```python
from build123d import *

# Parameters (mm, degrees)
BOSS_EXTRUDE1_DEPTH      = 10
BOSS_EXTRUDE2_DEPTH      = 10
BOSS_EXTRUDE2_DEPTH_BACK = 26
SKETCH2_R                = 5.820264096
CUT_EXTRUDE1_DEPTH       = 629.17046577
CUT_EXTRUDE1_DEPTH_BACK  = 629.17046577
SKETCH3_R                = 7.5


with BuildPart() as part:
    # Sketch1 → Boss-Extrude1 (new body)
    with BuildSketch(Plane.XY):
        with BuildLine():
            Line((-267.317020812, 384.57192575), (-267.301609192, 354.315771574))
            ThreePointArc((-267.301609192, 354.315771574), (-464.45214838, 194.902560898), (-291.585214163, 9.435771703))
            Line((-291.585214163, 9.435771703), (-291.585214163, -20.564228297))
            ThreePointArc((-291.585214163, -20.564228297), (-494.516390011, 194.886544), (-267.317020812, 384.57192575))
        make_face()
    extrude(amount=-BOSS_EXTRUDE1_DEPTH)

    # Sketch2 → Boss-Extrude2 (add, two sides: drawn at the far end of the back side and taken through both)
    with BuildSketch(Plane.XY.offset(-BOSS_EXTRUDE2_DEPTH_BACK)):
        with Locations((-307.201523558, -4.519874966)):
            Circle(SKETCH2_R)
    extrude(amount=BOSS_EXTRUDE2_DEPTH + BOSS_EXTRUDE2_DEPTH_BACK)

    # Sketch3 → Cut-Extrude1 (cut, two sides: drawn at the far end of the back side and taken through both)
    with BuildSketch(Plane.XY.offset(-CUT_EXTRUDE1_DEPTH_BACK)):
        with Locations(Location((-421.223956701, 321.632808197, 0), (0, 0, 180))):
            Circle(SKETCH3_R)
        with Locations(Location((-353.128945359, 362.487113382, 0), (0, 0, 180))):
            Circle(SKETCH3_R)
        with BuildLine():
            ThreePointArc((-374.845259184, 361.822893879), (-393.201425865, 352.083570004), (-410.432690408, 340.469492039))
            ThreePointArc((-410.432690408, 340.469492039), (-411.909575924, 329.966215923), (-401.406299807, 328.489330407))
            ThreePointArc((-401.406299807, 328.489330407), (-385.4837389, 339.221326502), (-368.521711461, 348.220954892))
            ThreePointArc((-368.521711461, 348.220954892), (-364.882515829, 358.183698247), (-374.845259184, 361.822893879))
        make_face()
    extrude(amount=CUT_EXTRUDE1_DEPTH + CUT_EXTRUDE1_DEPTH_BACK, mode=Mode.SUBTRACT)


solid = part.part
```
Model file for the job. Use its own axes, mm. A direction names the side the tool comes from. Coordinates: 2 decimals unless noted, no trailing zeros. Loops run counter-clockwise (first coordinate to the right, second up) from the corner with the lowest first, then second, coordinate; pieces in that order, holes last. Notation, with made-up numbers: (36, 38) - (95, 38) arc R24 cw to (95, 52) - close; hole circle Ø7 at (66.25, -23.75). An arc over 180 degrees is marked (long way). Answer as a JSON object with one key per item and string values. Group by question number.
(1) Tool access for faces 5 (the face through (-291.585, -5, -5)), 6 (the face through (-385.714, 339.083, -5.07)), 7 (the face through (-313, -4, -18)): list every direction of +Z, -Z, +X, -X, +Y, -Y with a clear straight run to the whole face (end or side of a thin tool).
(2) Two-plate mould, pull along Y, no slides. Class faces 1 (the face through (-392.952, 352.233, -5.07)), 2 (the face through (-465, 169, -10)), 3 (the face through (-412.01, 330.1, -5.07)), 4 (the face through (-313, -4, 5)): released by +Y, released by -Y, zero draft, split by the parting line, or undercut.
(3) Cut at C-C (y = 303.5). Give the cut face in (x, z), then the cut area to 3 significant figures.
(4) Probe line 1 along Y through (x, z) = (-348, -7) (3 decimals); line 2 along Y through (x, z) = (-342, -3); line 3 along X through (y, z) = (333, -4). List the from-to ranges inside material, lowest first.
(5) Cut at A-A (x = -386.5). Give the cut face in (y, z), then the cut area to 3 significant figures.
(6) Cut at B-B (x = -444). Give the cut face in (y, z).
(7) Cut at D-D (z = -14). Give the cut face in (x, y).
(8) Flat gauge pins, fed straight in: pin 1 (24 mm diameter, centred on x = -421.22, y = 321.63, fed in from +Z); pin 2 (10 mm diameter, centred on x = -385.5, z = 0.5, fed in from -Y); pin 3 (12 mm diameter, centred on x = -411.5, z = -11.5, fed in from -Y). Where does each tip first touch, or does it go through?
Geometry says:
{
 "1": {"face 5": "+Z, -Z, +X, -Y", "face 6": "+Z, -Z", "face 7": "-Z"},
 "2": {"face 1": "undercut", "face 2": "zero draft", "face 3": "undercut", "face 4": "split by the parting line"},
 "3": {"outline": "(-455.12, -10) - (-415.87, -10) - (-415.87, 0) - (-455.12, 0) - close", "area": "393 mm^2"},
 "4": {"line 1": "y = -12.58 to 18.876, 346.586 to 357.015, 367.959 to 378.041", "line 2": "y = -14.21 to 16.93, 348.53 to 379.68", "line 3": "x = -428.51 to -413.27, -395.15 to -377.9"},
 "5": {"outline": "(2.95, -10) - (37.74, -10) - (37.74, 0) - (2.95, 0) - close; (327.72, -10) - (338.61, -10) - (338.61, 0) - (327.72, 0) - close; (355.93, -10) - (362.51, -10) - (362.51, 0) - (355.93, 0) - close", "area": "523 mm^2"},
 "6": {"outline": "(48.2, -10) - (100.26, -10) - (100.26, 0) - (48.2, 0) - close; (265.2, -10) - (317.26, -10) - (317.26, 0) - (265.2, 0) - close"},
 "7": {"outline": "circle Ø11.64 at (-307.2, -4.52)"},
 "8": {"pin 1": "stops at z = 0", "pin 2": "stops at y = -0.08", "pin 3": "stops at y = 14.48"}
}
